```python
from build123d import *

# Parameters (mm, degrees)
SKETCH_1_W          = 84
SKETCH_1_H          = 10
SKETCH_2_W          = 45
SKETCH_2_H          = 40.446231626
CUT_EXTRUDE_1_DEPTH = 2
SWEEP_1_PROFILE_R   = 5


with BuildPart() as part:
    # 草图1 → 旋转1 (revolve)
    with BuildSketch(Plane.XY, mode=Mode.PRIVATE) as revolve_1_sk:
        with Locations((0, 5)):
            Rectangle(SKETCH_1_W, SKETCH_1_H)
    revolve(revolve_1_sk.sketch.rotate(Axis((-42, 0, 0), (1, 0, 0)), 180), axis=Axis((-42, 0, 0), (1, 0, 0)))

    # 草图2 → 切除-拉伸1 (cut)
    with BuildSketch(Plane(origin=(0, 10, 0), x_dir=(1, 0, 0), z_dir=(0, 1, 0))):
        with Locations((14.5, -3.02134906)):
            Rectangle(SKETCH_2_W, SKETCH_2_H)
    extrude(amount=-CUT_EXTRUDE_1_DEPTH, mode=Mode.SUBTRACT)

    # 扫描1: sweep along a path in 草图3
    with BuildLine(Plane.XY) as sweep_1_path:
        Line((42, 0), (55.00002565, 0))
        ThreePointArc((55.00002565, 0), (66.683449814, -11.683424164), (55.00002565, -23.366848328))
        Line((55.00002565, -23.366848328), (22.334289366, -23.366848328))
    # 扫描1 profile (on start of the path) → 扫描1 (sweep)
    with BuildSketch(Plane.YZ.offset(42)):
        Circle(SWEEP_1_PROFILE_R)
    sweep(path=sweep_1_path.line)


solid = part.part
```
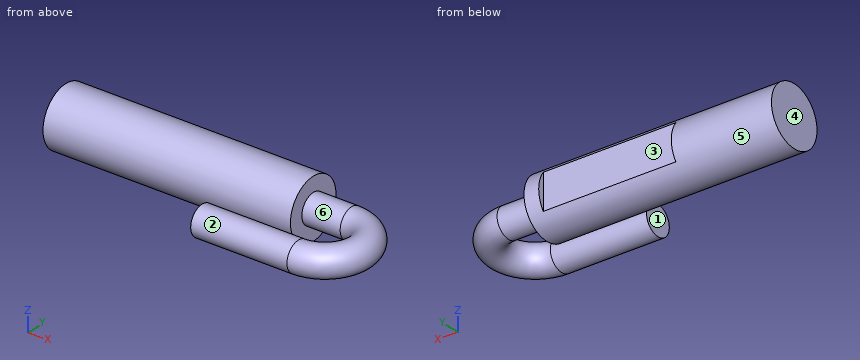
Part model, mm, in its own coordinate system. Face numbers are marked on the shaded views. A direction names the side the tool comes from. Round coordinates to 2 decimals unless told otherwise and drop trailing zeros. Loops run counter-clockwise (first coordinate to the right, second up) from the corner with the lowest first, then second, coordinate; pieces in that order, holes last.
1. 3-axis set-ups, long thin cutter, end or side, ignore diameter. For the marked faces 4, 5 and 6: which of +Z, -Z, +X, -X, +Y, -Y reach the whole face in a straight line?
Solutions:
face 4: +Z, -Z, -X, +Y, -Y
face 5: -X
face 6: none
2. Slice it at C-C (x = 20.5). Give the cut face in (y, z), and give its area (3 significant figures).
Solutions:
outline: (8, -6) - (8, 6) arc R10 ccw (long way) to start
area: 298 mm2
3. Two-plate mould, pull along X, no slides. Class the marked faces 1, 2 and 3: pulls with the +X half, pulls with the -X half, needs draft (parallel to the pull), parting line crosses it, or undercut.
Solutions:
face 1: pulls with the -X half
face 2: needs draft
face 3: undercut
4. Slice it at A-A (z = 0). Give the cut face in (x, y), and give its area (3 significant figures).
Solutions:
outline: (-42, -10) - (42, -10) - (42, -5) - (55, -5) arc R6.68 cw to (55, -18.37) - (22.33, -18.37) - (22.33, -28.37) - (55, -28.37) arc R16.68 ccw to (55, 5) - (42, 5) - (42, 10) - (37, 10) - (37, 8) - (-8, 8) - (-8, 10) - (-42, 10) - close
area: 2,410 mm2
5. Slice it at B-B (x = 49). Give the cut face in (y, z).
Solutions:
outline: circle Ø10 at (-23.37, 0); circle Ø10 at (0, 0)
6. Flat gauge pins, fed straight in: pin 1 (6 mm diameter, centred on y = 2, z = -2, fed in from +X); pin 2 (1.6 mm diameter, centred on y = 8.5, z = 1.5, fed in from +X); pin 3 (2 mm diameter, centred on x = 33, z = 3, fed in from -Y). Where does each tip first touch, or does it go through?
Solutions:
pin 1: stops at x = 67.54
pin 2: stops at x = 42
pin 3: stops at y = -27.95
7. Drill centre lines: line 1 along Z through (x, y) = (33, -0.5); line 2 along Y through (x, z) = (8.5, -8); line 3 along X through (y, z) = (-0.5, 5.25). Where is each one in solid material? Low to high.
Solutions:
line 1: z = -9.99 to 9.99
line 2: y = -6 to 6
line 3: x = -42 to 42
8. Slice it at D-D (z = -8.5). Give the cut face in (x, y), and give its area (3 significant figures).
Solutions:
outline: (-42, -5.27) - (42, -5.27) - (42, 5.27) - (-42, 5.27) - close
area: 885 mm2
